Geometry: final body of the model. Coordinates: model frame, mm. Face numbers are marked on the shaded views. A direction names the side the tool comes from. Give positions to 0.01 mm unless a question says otherwise; leave off trailing zeros. Write each loop counter-clockwise with the first axis right and the second up, starting at its lowest first coordinate (ties: lowest second). Pieces come first, ordered by that corner, then holes. Notation, with made-up numbers: (29.25, -8) - (64.25, -8) arc R26 cw to (64.25, 7) - close; hole circle Ø10 at (4.25, 8.5). An arc over 180 degrees is marked (long way). Return JSON: item names as keys, results as strings.
from build123d import *

# Parameters (mm, degrees)
BASE_PLATE_SKETCH_R   = 4
BASE_PLATE_DEPTH      = 5
LUG_PROFILE_SKETCH_R  = 4
LUG_SUPPORT_WEB_DEPTH = 4.5
LUG_EYE_DEPTH         = 9


with BuildPart() as part:
    # Base Plate Sketch → Base Plate (new body)
    with BuildSketch(Plane.XY):
        with BuildLine():
            Line((-22, -15), (22, -15))
            ThreePointArc((22, -15), (27.656854249, -12.656854249), (30, -7))
            Line((30, -7), (30, 7))
            ThreePointArc((30, 7), (27.656854249, 12.656854249), (22, 15))
            Line((22, 15), (-22, 15))
            ThreePointArc((-22, 15), (-27.656854249, 12.656854249), (-30, 7))
            Line((-30, 7), (-30, -7))
            ThreePointArc((-30, -7), (-27.656854249, -12.656854249), (-22, -15))
        make_face()
        with Locations((20, 0)):
            Circle(BASE_PLATE_SKETCH_R, mode=Mode.SUBTRACT)
        with Locations((-20, 0)):
            Circle(BASE_PLATE_SKETCH_R, mode=Mode.SUBTRACT)
    extrude(amount=BASE_PLATE_DEPTH)



with BuildPart() as body_2:
    # Lug Profile Sketch → Lug Support Web (new, symmetric)
    with BuildSketch(Plane(origin=(0, 0, 0), x_dir=(0, 0, -1), z_dir=(1, 0, 0))):
        with BuildLine():
            ThreePointArc((-32.17423683, 4.289332839), (-33.028883618, 6.27753657), (-31.573908753, 7.87954261))
            Line((-31.573908753, 7.87954261), (-43.235238064, 4.754898838))
            ThreePointArc((-43.235238064, 4.754898838), (-52.086936749, -10.506015692), (-36.861605806, -19.418780673))
            Line((-36.861605806, -19.418780673), (-36.668125757, -19.36693785))
            Line((-36.668125757, -19.36693785), (-20.370491826, -15))
            Line((-20.370491826, -15), (-25.04245288, -15))
            ThreePointArc((-25.04245288, -15), (-26.688692003, -14.135736214), (-26.91214627, -12.289896749))
            ThreePointArc((-26.91214627, -12.289896749), (-26.655991742, -3.083912061), (-32.17423683, 4.289332839))
        make_face()
        with Locations((-40, -7.31917399)):
            Circle(LUG_PROFILE_SKETCH_R, mode=Mode.SUBTRACT)
    extrude(amount=LUG_SUPPORT_WEB_DEPTH, both=True)


with BuildPart() as part_1:
    add(part.part)

    add(body_2.part)  # Lug Eye merges body 2
    # Sketch4_3 → Lug Eye (add, symmetric)
    with BuildSketch(Plane(origin=(0, 0, 0), x_dir=(0, 0, -1), z_dir=(1, 0, 0))):
        with BuildLine():
            Line((-5, -15), (-5, 15))
            Line((-5, 15), (-31.573908753, 7.87954261))
            ThreePointArc((-31.573908753, 7.87954261), (-33.028883618, 6.27753657), (-32.17423683, 4.289332839))
            ThreePointArc((-32.17423683, 4.289332839), (-26.655991742, -3.083912061), (-26.91214627, -12.289896749))
            ThreePointArc((-26.91214627, -12.289896749), (-26.688692003, -14.135736214), (-25.04245288, -15))
            Line((-25.04245288, -15), (-20.370491826, -15))
            Line((-20.370491826, -15), (-5, -15))
        make_face()
    extrude(amount=LUG_EYE_DEPTH, both=True)


solid = part_1.part
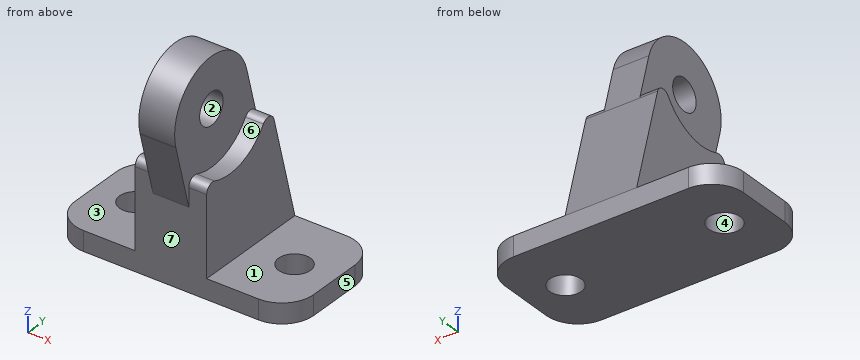
Q1. Pin query (flat end, axial travel): P1, Ø8.5, axis at y = 2.5, z = 20.5, coming from the +X side; P2, Ø20, axis at x = 6, z = 10, coming from the -Y side; P3, Ø8.5, axis at y = -6.5, z = 36, coming from the +X side. Return the tip coordinate at first contact, or that it passes through.
Answer key:
{"P1": "stops at x = 9", "P2": "stops at y = -15", "P3": "stops at x = 4.5"}
Q2. Set-up query: the marked faces 1, 2 and 3. Return all of +Z, -Z, +X, -X, +Y, -Y with unobstructed straight access to the full face (end or side cutting, diameter ignored); none if empty.
Answer key:
{"face 1": "+Z, +X, +Y, -Y", "face 2": "+X, -X", "face 3": "+Z, -X, +Y, -Y"}
Q3. Mould query, pull axis Y, two halves, no side actions, for the marked faces 4, 5, 6 and 7. Classes: pulls with the +Y half, pulls with the -Y half, needs draft (parallel to the pull), parting line crosses it, or undercut.
Answer key:
{"face 4": "undercut", "face 5": "needs draft", "face 6": "undercut", "face 7": "pulls with the -Y half"}
Q4. Section query A-A, the plane x = -20. Return the cut outline in (y, z).
Answer key:
{"outline": "(-15, 0) - (-4, 0) - (-4, 5) - (-15, 5) - close; (4, 0) - (15, 0) - (15, 5) - (4, 5) - close"}
Q5. Section query C-C, the plane y = -8.5. Return the cut outline in (x, z), plus the area to 3 significant figures.
Answer key:
{"outline": "(-29.86, 0) - (29.86, 0) - (29.86, 5) - (9, 5) - (9, 26.05) - (4.5, 26.05) - (4.5, 36.18) - (-4.5, 36.18) - (-4.5, 26.05) - (-9, 26.05) - (-9, 5) - (-29.86, 5) - close; (-4.5, 43.82) - (4.5, 43.82) - (4.5, 52.44) - (-4.5, 52.44) - close", "area": "846 mm^2"}
Q6. Material intervals for probe 1 along Y at (x, z) = (-20, 1.75); probe 2 along X at (y, z) = (-3.5, 41.5); probe 3 along Y at (x, z) = (-4, 39.5), sorted ascending. Write a range as [from, to].
Answer key:
{"probe 1": "y = [-15, -4], [4, 15]", "probe 2": "x = [-4.5, 4.5]", "probe 3": "y = [-19.81, -11.29], [-3.35, 5.76]"}
Q7. Section query D-D, the plane y = 0. Return the cut outline in (x, z).
Answer key:
{"outline": "(-30, 0) - (-24, 0) - (-24, 5) - (-30, 5) - close; (-16, 0) - (16, 0) - (16, 5) - (9, 5) - (9, 28.07) - (4.5, 28.07) - (4.5, 50.13) - (-4.5, 50.13) - (-4.5, 28.07) - (-9, 28.07) - (-9, 5) - (-16, 5) - close; (24, 0) - (30, 0) - (30, 5) - (24, 5) - close"}
Q8. Section query B-B, the plane z = 38.5. Return the cut outline in (x, y), plus the area to 3 significant figures.
Answer key:
{"outline": "(-4.5, -19.73) - (4.5, -19.73) - (4.5, -11.03) - (-4.5, -11.03) - close; (-4.5, -3.61) - (4.5, -3.61) - (4.5, 6.02) - (-4.5, 6.02) - close", "area": "165 mm^2"}
